Verification items for the finished model (mm, model axes). A direction names the side the tool comes from. Round coordinates to 2 decimals unless told otherwise and drop trailing zeros. Write each loop counter-clockwise with the first axis right and the second up, starting at its lowest first coordinate (ties: lowest second). Pieces come first, ordered by that corner, then holes.
from build123d import *
from build123d.topology import SkipClean

# Parameters (mm, degrees)
SKETCH_1_R        = 34
SKETCH_1_R_2      = 29
EXTRUDE_1_DEPTH   = 60
EXTRUDE_1_2_DEPTH = 60
EXTRUDE_START     = -60
EXTRUDE_2_DEPTH   = 60
EXTRUDE_START_2   = -2
SKETCH_4_R        = 34
EXTRUDE_3_DEPTH   = 2


with BuildPart() as part:
    # Sketch 1 → Extrude 1 (new body)
    with BuildSketch(Plane.XY):
        Circle(SKETCH_1_R)
        Circle(SKETCH_1_R_2, mode=Mode.SUBTRACT)
    extrude(amount=EXTRUDE_1_DEPTH)



with BuildPart() as body_2:
    # Sketch 1 → Extrude 1 2 (new body)
    with BuildSketch(Plane.XY):
        Polygon((-15, 0.078188502), (-7.567713229, -12.951286806), (7.432286771, -13.029475308), (15, -0.078188502), (7.567713229, 12.951286806), (-7.432286771, 13.029475308), align=None)
        with BuildLine():
            ThreePointArc((-10.461357464, 4), (-11.2, 0), (-10.461357464, -4))
            Line((-10.461357464, -4), (-7.5, -4))
            ThreePointArc((-7.5, -4), (-6.01040764, -6.01040764), (-4, -7.5))
            Line((-4, -7.5), (-4, -10.461357464))
            ThreePointArc((-4, -10.461357464), (0, -11.2), (4, -10.461357464))
            Line((4, -10.461357464), (4, -7.5))
            ThreePointArc((4, -7.5), (6.01040764, -6.01040764), (7.5, -4))
            Line((7.5, -4), (10.461357464, -4))
            ThreePointArc((10.461357464, -4), (11.2, 0), (10.461357464, 4))
            Line((10.461357464, 4), (7.5, 4))
            ThreePointArc((7.5, 4), (6.01040764, 6.01040764), (4, 7.5))
            Line((4, 7.5), (4, 10.461357464))
            ThreePointArc((4, 10.461357464), (0, 11.2), (-4, 10.461357464))
            Line((-4, 10.461357464), (-4, 7.5))
            ThreePointArc((-4, 7.5), (-6.01040764, 6.01040764), (-7.5, 4))
            Line((-7.5, 4), (-10.461357464, 4))
        make_face(mode=Mode.SUBTRACT)
    extrude(amount=EXTRUDE_1_2_DEPTH)


with BuildPart() as part_1:
    add(part.part)

    add(body_2.part)  # Extrude 2 merges body 2
    # Sketch 2 → Extrude 2 (add)
    with BuildSketch(Plane.XY.offset(EXTRUDE_START)):
        with BuildLine():
            ThreePointArc((16.926969134, 29.486907535), (14.75204713, 30.632941509), (12.5, 31.618823508))
            ThreePointArc((12.5, 31.618823508), (0, 20), (-12.5, 31.618823508))
            ThreePointArc((-12.5, 31.618823508), (-14.75204713, 30.632941509), (-16.926969134, 29.486907535))
            ThreePointArc((-16.926969134, 29.486907535), (-15.636629649, 12.469796037), (-32.51421418, 9.941120473))
            ThreePointArc((-32.51421418, 9.941120473), (-33.147549014, 7.565711755), (-33.607585262, 5.150748765))
            ThreePointArc((-33.607585262, 5.150748765), (-19.498558244, -4.450418679), (-28.044561913, -19.22244904))
            ThreePointArc((-28.044561913, -19.22244904), (-26.582270404, -21.198653263), (-24.981004219, -23.064028881))
            ThreePointArc((-24.981004219, -23.064028881), (-8.677674782, -18.019377358), (-2.456782521, -33.911122359))
            ThreePointArc((-2.456782521, -33.911122359), (0, -34), (2.456782521, -33.911122359))
            ThreePointArc((2.456782521, -33.911122359), (8.677674782, -18.019377358), (24.981004219, -23.064028881))
            ThreePointArc((24.981004219, -23.064028881), (26.582270404, -21.198653263), (28.044561913, -19.22244904))
            ThreePointArc((28.044561913, -19.22244904), (19.498558244, -4.450418679), (33.607585262, 5.150748765))
            ThreePointArc((33.607585262, 5.150748765), (33.147549014, 7.565711755), (32.51421418, 9.941120473))
            ThreePointArc((32.51421418, 9.941120473), (15.636629649, 12.469796037), (16.926969134, 29.486907535))
        make_face()
        with BuildLine():
            Line((-10.461357464, -4), (-7.5, -4))
            ThreePointArc((-7.5, -4), (-6.01040764, -6.01040764), (-4, -7.5))
            Line((-4, -7.5), (-4, -10.461357464))
            ThreePointArc((-4, -10.461357464), (0, -11.2), (4, -10.461357464))
            Line((4, -10.461357464), (4, -7.5))
            ThreePointArc((4, -7.5), (6.01040764, -6.01040764), (7.5, -4))
            Line((7.5, -4), (10.461357464, -4))
            ThreePointArc((10.461357464, -4), (11.2, 0), (10.461357464, 4))
            Line((10.461357464, 4), (7.5, 4))
            ThreePointArc((7.5, 4), (6.01040764, 6.01040764), (4, 7.5))
            Line((4, 7.5), (4, 10.461357464))
            ThreePointArc((4, 10.461357464), (0, 11.2), (-4, 10.461357464))
            Line((-4, 10.461357464), (-4, 7.5))
            ThreePointArc((-4, 7.5), (-6.01040764, 6.01040764), (-7.5, 4))
            Line((-7.5, 4), (-10.461357464, 4))
            ThreePointArc((-10.461357464, 4), (-11.2, 0), (-10.461357464, -4))
        make_face(mode=Mode.SUBTRACT)
    extrude(amount=EXTRUDE_2_DEPTH)

    # Sketch 4 → Extrude 3 (add)
    with SkipClean():  # the faces are left unmerged after this step: merging them gives an invalid solid
        with BuildSketch(Plane.XY.offset(EXTRUDE_START_2)):
            with Locations(Location((0, 0, 0), (0, 0, 171.286564556))):
                Circle(SKETCH_4_R)
            with BuildLine():
                ThreePointArc((21.649435664, -19.295127245), (22.673112992, -18.081204254), (23.628810764, -16.813069377))
                ThreePointArc((23.628810764, -16.813069377), (19.498558244, -4.450418679), (28.583740291, 4.895895317))
                ThreePointArc((28.583740291, 4.895895317), (28.272909453, 6.453107085), (27.877309497, 7.990970854))
                ThreePointArc((27.877309497, 7.990970854), (15.636629649, 12.469796037), (13.993905477, 25.400208848))
                ThreePointArc((13.993905477, 25.400208848), (12.582628434, 26.128097169), (11.133625585, 26.777647046))
                ThreePointArc((11.133625585, 26.777647046), (0, 20), (-11.133625585, 26.777647046))
                ThreePointArc((-11.133625585, 26.777647046), (-12.582628434, 26.128097169), (-13.993905477, 25.400208848))
                ThreePointArc((-13.993905477, 25.400208848), (-15.636629649, 12.469796037), (-27.877309497, 7.990970854))
                ThreePointArc((-27.877309497, 7.990970854), (-28.272909453, 6.453107085), (-28.583740291, 4.895895317))
                ThreePointArc((-28.583740291, 4.895895317), (-19.498558244, -4.450418679), (-23.628810764, -16.813069377))
                ThreePointArc((-23.628810764, -16.813069377), (-22.673112992, -18.081204254), (-21.649435664, -19.295127245))
                ThreePointArc((-21.649435664, -19.295127245), (-8.677674782, -18.019377358), (-1.587335586, -28.956525443))
                ThreePointArc((-1.587335586, -28.956525443), (0, -29), (1.587335586, -28.956525443))
                ThreePointArc((1.587335586, -28.956525443), (8.677674782, -18.019377358), (21.649435664, -19.295127245))
            make_face(mode=Mode.SUBTRACT)
        extrude(amount=EXTRUDE_3_DEPTH)


solid = part_1.part
Q1. Tool access check on faces 1 (the flat face through (9, 4, -1)), 2 (the cylindrical face through (15.8, 12.27, -31.41)), 3 (the flat face through (11.336, 6.345, 29.58)). Record the directions out of +Z, -Z, +X, -X, +Y, -Y that give a thin tool (end or side, any length) a straight path to the whole face; none if there is none.
Recorded:
face 1: +Z, -Z
face 2: -Z
face 3: +Z
Q2. Sectioned sample at B-B (x = 0). Enter the section's corners in (y, z), plus the area to 3 significant figures.
Recorded:
outline: (-34, -60) - (-11.2, -60) - (-11.2, 60) - (-12.99, 60) - (-12.99, 0) - (-29, 0) - (-29, 60) - (-34, 60) - close; (11.2, -60) - (20, -60) - (20, -2) - (34, -2) - (34, 60) - (29, 60) - (29, 0) - (12.99, 0) - (12.99, 60) - (11.2, 60) - close
area: 2,740 mm2
Q3. Depth check by flat-ended pin: P1, Ø7.5, axis at x = 20.5, y = 16.5, coming from the +Z side; P2, Ø0.9, axis at y = -9, z = 10, coming from the -X side; P3, Ø2.5, axis at x = -9, z = 17, coming from the -Y side; P4, Ø3, axis at x = -23.5, y = -6.5, coming from the +Z side. Enter the tip coordinate at first touch or a pass-through.
Recorded:
P1: stops at z = 60
P2: stops at x = -32.91
P3: stops at y = -33.1
P4: stops at z = 0
Q4. Material ranges on line 1 along Y through (x, z) = (0, 43); line 2 along X through (y, z) = (0, 37); line 3 along X through (y, z) = (-10, 53.5), recorded low to high.
Recorded:
line 1: y = -34 to -29, -12.99 to -11.2, 11.2 to 12.99, 29 to 34
line 2: x = -34 to -29, -14.96 to -11.2, 11.2 to 14.96, 29 to 34
line 3: x = -32.5 to -27.22, -9.25 to -4, 4 to 9.2, 27.22 to 32.5
Q5. Sectioned sample at A-A (z = 11.5). Enter the section's corners in (x, y).
Recorded:
outline: circle Ø68 at (0, 0); (-15, 0.08) - (-7.57, -12.95) - (7.43, -13.03) - (15, -0.08) - (7.57, 12.95) - (-7.43, 13.03) - close; hole circle Ø58 at (0, 0); hole (-10.46, -4) - (-7.5, -4) arc R8.5 ccw to (-4, -7.5) - (-4, -10.46) arc R11.2 ccw to (4, -10.46) - (4, -7.5) arc R8.5 ccw to (7.5, -4) - (10.46, -4) arc R11.2 ccw to (10.46, 4) - (7.5, 4) arc R8.5 ccw to (4, 7.5) - (4, 10.46) arc R11.2 ccw to (-4, 10.46) - (-4, 7.5) arc R8.5 ccw to (-7.5, 4) - (-10.46, 4) arc R11.2 ccw to start
Q6. Release check for a two-part mould opening along Y. For faces 4 (the flat face through (4, -9, -1)), 5 (the flat face through (7, 7, -60)) record: released by +Y, released by -Y, zero draft, split by the parting line, or undercut.
Recorded:
face 4: undercut
face 5: zero draft
